For this review, take the finished solid that the model builds, in its own axes (mm). A direction names the side the tool comes from. Give positions to 0.01 mm unless a question says otherwise; leave off trailing zeros. Order: outer loops, then holes, each group sorted by start corner. A loop starts at its lowest first (then second) coordinate and runs counter-clockwise, first axis right, second up. Notation, with made-up numbers: (5.25, 35) - (18.25, 35) arc R21 cw to (18.25, 49) - close; hole circle Ø5 at (83.5, 51.25). An arc over 180 degrees is marked (long way). Use a Markdown table: item, result. Add a question column.
1) We need section A-A on x = 0. Write out the cut boundary in (y, z).
2) Machinability: for faces 1 (the face through (2, -7, 0)), 2 (the face through (0.9, 0.49, 2.86)), which of the approach directions +Z, -Z, +X, -X, +Y, -Y give a long, thin tool a straight path to every point of the face, cutting with its end or side? Answer none if there is none.
3) Wall thickness on L1, parallel to Z at x = 0.75, y = -8; L2, parallel to Y at x = 0.1, z = -2.45; L3, parallel to X at y = -3, z = 1.7: over which ranges is each line inside the solid? List them lowest first.
4) Mouldability with a two-part tool opening along Y and no side actions: class faces 3 (the face through (0, 1.5, 0)), 4 (the face through (-1, 0, 2)), 5 (the face through (2, -17, 0)), 6 (the face through (1.806, -15.394, 0.401)) as released by +Y, released by -Y, zero draft, split by the parting line, or undercut.
5) We need section B-B on z = 0. Write out the cut boundary in (x, y), then the cut area to 3 significant figures.
6) We need section C-C on y = -3.5. Write out the cut boundary in (x, z), then the cut area to 3 significant figures.
7) Clearance check with flat-ended pins moving along their axes: P1, Ø1.5, axis at y = -1, z = 2.5, coming from the -X side; P2, Ø3, axis at y = -8, z = -1.5, coming from the +X side. State where each tip first meets the part, or that it passes through.
```python
from build123d import *

# Parameters (mm, degrees)
SKETCH1_R           = 3
BOSS_EXTRUDE1_DEPTH = 1.5
SKETCH2_R           = 2
BOSS_EXTRUDE2_DEPTH = 18
SKETCH3_W           = 0.15
SKETCH3_H           = 0.8
CHAMFER1_SIZE       = 0.5


with BuildPart() as part:
    # Sketch1 → Boss-Extrude1 (new body)
    with BuildSketch(Plane(origin=(0, 0, 0), x_dir=(1, 0, 0), z_dir=(0, 1, 0))):
        with Locations(Location((0, 0, 0), (0, 0, 270))):
            Circle(SKETCH1_R)
    extrude(amount=BOSS_EXTRUDE1_DEPTH)

    # Sketch2 → Boss-Extrude2 (add)
    with BuildSketch(Plane.XZ):
        with Locations(Location((0, 0, 0), (0, 0, 90))):
            Circle(SKETCH2_R)
    extrude(amount=BOSS_EXTRUDE2_DEPTH)

    # Sketch3 → Cut-Revolve1 (revolve, cut)
    with BuildSketch(Plane(origin=(0, 0, 0), x_dir=(0, 0, -1), z_dir=(1, 0, 0))):
        with Locations((1.925, -15.4)):
            Rectangle(SKETCH3_W, SKETCH3_H)
    revolve(axis=Axis((0, -16.563495901, 0), (0, 1, 0)), mode=Mode.SUBTRACT)

    # Chamfer1
    chamfer1_edges = [part.edges().sort_by_distance(p)[0] for p in [
        (0, 1.5, -3),
        (0, -18, -2),
    ]]
    chamfer(chamfer1_edges, length=CHAMFER1_SIZE)


solid = part.part
```
Checked values:
| question | item | result |
|---|---|---|
| 1 | outline | (-18, -1.5) - (-17.5, -2) - (-15.8, -2) - (-15.8, -1.85) - (-15, -1.85) - (-15, -2) - (0, -2) - (0, -3) - (1, -3) - (1.5, -2.5) - (1.5, 2.5) - (1, 3) - (0, 3) - (0, 2) - (-15, 2) - (-15, 1.85) - (-15.8, 1.85) - (-15.8, 2) - (-17.5, 2) - (-18, 1.5) - close |
| 2 | face 1 | -Y |
| 2 | face 2 | +Y, -Y |
| 3 | L1 | -1.85 to 1.85 |
| 3 | L2 | 0 to 1.5 |
| 3 | L3 | -1.05 to 1.05 |
| 4 | face 3 | released by +Y |
| 4 | face 4 | released by -Y |
| 4 | face 5 | zero draft |
| 4 | face 6 | undercut |
| 5 | outline | (-3, 0) - (-2, 0) - (-2, -15) - (-1.85, -15) - (-1.85, -15.8) - (-2, -15.8) - (-2, -17.5) - (-1.5, -18) - (1.5, -18) - (2, -17.5) - (2, -15.8) - (1.85, -15.8) - (1.85, -15) - (2, -15) - (2, 0) - (3, 0) - (3, 1) - (2.5, 1.5) - (-2.5, 1.5) - (-3, 1) - close |
| 5 | area | 80.3 mm² |
| 6 | outline | circle Ø4 at (0, 0) |
| 6 | area | 12.6 mm² |
| 7 | P1 | x = -0.97 |
| 7 | P2 | x = 2 |
